Verification items for the finished model (mm, model axes). Round coordinates to 2 decimals unless told otherwise and drop trailing zeros. Loops run counter-clockwise (first coordinate to the right, second up) from the corner with the lowest first, then second, coordinate; pieces in that order, holes last. Notation, with made-up numbers: (-15.75, 30) -> (16.25, 30) arc R20 cw to (16.25, 34) -> close; hole circle Ø5 at (34.25, 50.25). An arc over 180 degrees is marked (long way). Write item = value, one per line.
```python
from build123d import *

# Parameters (mm, degrees)
SKETCH1_R             = 11
BOSS_EXTRUDE1_DEPTH   = 100
SKETCH2_R             = 3
BOSS_EXTRUDE2_DEPTH   = 5
SKETCH3_R             = 1.85
CUT_EXTRUDE1_DEPTH    = 107.146125695
SKETCH4_R             = 3
CUT_EXTRUDE2_DEPTH    = 102.202766761
M6_TAPPED_HOLE1_D     = 5
M6_TAPPED_HOLE1_DEPTH = 10
M6_TAPPED_HOLE1_TIP   = 1.502151548
CHAMFER1_SIZE         = 0.3


with BuildPart() as part:
    # Sketch1 → Boss-Extrude1 (new body)
    with BuildSketch(Plane.XY):
        Circle(SKETCH1_R)
    extrude(amount=BOSS_EXTRUDE1_DEPTH)

    # Sketch2 → Boss-Extrude2 (add)
    with BuildSketch(Plane.XY.offset(100)):
        Circle(SKETCH2_R)
    extrude(amount=BOSS_EXTRUDE2_DEPTH)

    # Sketch3 → Cut-Extrude1 (cut, through all)
    with BuildSketch(Plane.XY.offset(105)):
        Circle(SKETCH3_R)
    extrude(amount=-CUT_EXTRUDE1_DEPTH, mode=Mode.SUBTRACT)

    # Sketch4 → Cut-Extrude2 (cut, through all)
    with BuildSketch(Plane.XY.offset(100)):
        with Locations((6.5, 0)):
            Circle(SKETCH4_R)
    extrude(amount=-CUT_EXTRUDE2_DEPTH, mode=Mode.SUBTRACT)

    # M6 Tapped Hole1
    with Locations(Plane.XY.offset(100)):
        with Locations((0, 7.5)):
            Hole(M6_TAPPED_HOLE1_D / 2, depth=M6_TAPPED_HOLE1_DEPTH)
            with Locations((0, 0, -(M6_TAPPED_HOLE1_DEPTH + M6_TAPPED_HOLE1_TIP / 2))):  # 118° drill point
                Cone(0, M6_TAPPED_HOLE1_D / 2, M6_TAPPED_HOLE1_TIP, mode=Mode.SUBTRACT)

    # Chamfer1
    chamfer1_edges = [part.edges().sort_by_distance(p)[0] for p in [
        (-1.85, 0, 0),
        (-1.85, 0, 105),
        (3.5, 0, 0),
        (3.5, 0, 100),
        (-11, 0, 0),
        (-11, 0, 100),
        (-3, 0, 105),
    ]]
    chamfer(chamfer1_edges, length=CHAMFER1_SIZE)


solid = part.part
```
(1) Sectioned sample at A-A, the plane y = 0. Count the separate pieces of the cut face and the enclosed holes in it, and give its area (3 significant figures).
Filled sheet:
separate_pieces = 3
enclosed_holes = 0
area = 1,240 mm2
(2) Sectioned sample at B-B, the plane z = 47.5. Record the cut outline in (x, y).
Filled sheet:
outline = circle Ø22 at (0, 0); hole circle Ø3.7 at (0, 0); hole circle Ø6 at (6.5, 0)
(3) Go/stop test with flat-tipped pins: pin 1 Ø8 at (x, y) = (0, 1.5) entering from -Z; pin 2 Ø5 at (x, z) = (4, 73.5) entering from +Y; pin 3 Ø2 at (x, z) = (-7, 56.5) entering from -Y; pin 4 Ø8 at (x, z) = (6.5, 32.5) entering from +Y. Record where each tip stops, or that it passes through.
Filled sheet:
pin_1 = 0
pin_2 = 10.9
pin_3 = -9.22
pin_4 = 10.71
(4) Material ranges on probe 1 along Y at (x, z) = (0, 96.25); probe 2 along Y at (x, z) = (0, 70); probe 3 along X at (y, z) = (2.5, 45.5), recorded low to high. Write a range as from..to.
Filled sheet:
probe_1 = -11..-1.85, 1.85..5, 10..11
probe_2 = -11..-1.85, 1.85..11
probe_3 = -10.71..4.84, 8.16..10.71
(5) Draft check along Y on faces 1 (the face through (0.54, 5.06, 94.93)), 2 (the face through (-3, -2, 100)), 3 (the face through (-3, 0, 102)), 4 (the face through (-0.401, -1.806, 53.231)). Enter one of: released by +Y, released by -Y, zero draft, split by the parting line, or undercut.
Filled sheet:
face_1 = undercut
face_2 = zero draft
face_3 = split by the parting line
face_4 = undercut
